Can you work these out from the model? Positions are in its coordinate system, mm. Face numbers are marked on the shaded views. Give positions to 0.01 mm unless a question says otherwise; leave off trailing zeros. Loops run counter-clockwise (first coordinate to the right, second up) from the corner with the lowest first, then second, coordinate; pieces in that order, holes last.
from build123d import *

# Parameters (mm, degrees)
BOSS_EXTRUDE1_DEPTH = 34
CHAMFER1_SIZE       = 1


with BuildPart() as part:
    # Sketch1 → Boss-Extrude1 (new body)
    with BuildSketch(Plane.XY):
        Polygon((-13.5, 5), (13.5, 5), (13.5, -5.5), (6, -5.5), (6, -4), (5, -3), (4, -3), (4, -2), (5, -2), (6, -1), (6, 0.5), (-6, 0.5), (-6, -1), (-5, -2), (-4, -2), (-4, -3), (-5, -3), (-6, -4), (-6, -5.5), (-13.5, -5.5), align=None)
    extrude(amount=BOSS_EXTRUDE1_DEPTH)

    # Chamfer1
    chamfer1_edges = [part.edges().sort_by_distance(p)[0] for p in [
        (-13.5, -5.5, 17),
        (-13.5, 5, 17),
        (13.5, 5, 17),
        (13.5, -5.5, 17),
    ]]
    chamfer(chamfer1_edges, length=CHAMFER1_SIZE)


solid = part.part
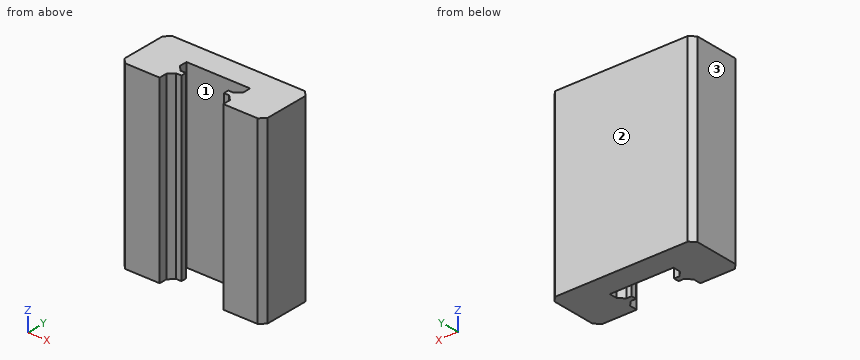
(1) Suppose I cut it at A-A on y = -1.5. List the corners of the cut face in (x, z) for me, plus the area to 3 significant figures.
Returned:
outline: (-13.5, 0) - (-5.5, 0) - (-5.5, 34) - (-13.5, 34) - close; (5.5, 0) - (13.5, 0) - (13.5, 34) - (5.5, 34) - close
area: 544 mm2
(2) Will these pins go through, and if not, where does the flat tip stop? P1, Ø0.5, axis at x = 4.5, z = 19.5, coming from the -Y side; P2, Ø0.8, axis at y = -5, z = 21.5, coming from the -X side; P3, Ø6, axis at x = 2.5, z = 22, coming from the -Y side.
Returned:
P1: stops at y = -3
P2: stops at x = -13.4
P3: stops at y = -3.5
(3) Suppose I cut it at D-D on x = 0.75. List the corners of the cut face in (y, z) for me.
Returned:
outline: (0.5, 0) - (5, 0) - (5, 34) - (0.5, 34) - close
(4) Suppose I cut it at C-C on y = -5. List the corners of the cut face in (x, z) for me.
Returned:
outline: (-13, 0) - (-6, 0) - (-6, 34) - (-13, 34) - close; (6, 0) - (13, 0) - (13, 34) - (6, 34) - close
(5) Thinking about a two-plate mould opening in X: for the marked faces 1, 2 and 3, which applies, pulls with the +X half, pulls with the -X half, needs draft (parallel to the pull), parting line crosses it, or undercut?
Returned:
face 1: undercut
face 2: needs draft
face 3: pulls with the -X half
(6) Please list where these lines run through material, in increasing order: probe 1 along X at (y, z) = (-2.75, 26.5); probe 2 along X at (y, z) = (-4, 15); probe 3 along Y at (x, z) = (-2, 15).
Returned:
probe 1: x = -13.5 to -4, 4 to 13.5
probe 2: x = -13.5 to -6, 6 to 13.5
probe 3: y = 0.5 to 5
(7) Suppose I cut it at B-B on z = 4. List the corners of the cut face in (x, y) for me.
Returned:
outline: (-13.5, -4.5) - (-12.5, -5.5) - (-6, -5.5) - (-6, -4) - (-5, -3) - (-4, -3) - (-4, -2) - (-5, -2) - (-6, -1) - (-6, 0.5) - (6, 0.5) - (6, -1) - (5, -2) - (4, -2) - (4, -3) - (5, -3) - (6, -4) - (6, -5.5) - (12.5, -5.5) - (13.5, -4.5) - (13.5, 4) - (12.5, 5) - (-12.5, 5) - (-13.5, 4) - close
